Geometry check sheet. Reference: the model listing, model coordinates, mm. A direction names the side the tool comes from. Give positions to 0.01 mm unless a question says otherwise; leave off trailing zeros. Write each loop counter-clockwise with the first axis right and the second up, starting at its lowest first coordinate (ties: lowest second). Pieces come first, ordered by that corner, then holes. Notation, with made-up numbers: (9.25, -7.5) -> (49.25, -7.5) arc R27 ccw to (49.25, 9.5) -> close; hole circle Ø1 at (52.25, -9.75). An arc over 180 degrees is marked (long way). Write item = value, one per line. Start each with the question number.
1. Mould release check, pull along Y, two halves, no side actions. Record for faces 1 (the cylindrical face through (-2.994, 22.804, 4.93)), 2 (the flat face through (-14.07, -24.83, -7.4)), 3 (the flat face through (22.1, -7.3, 10)): pulls with the +Y half, pulls with the -Y half, needs draft (parallel to the pull), parting line crosses it, or undercut.
2. Depth check by flat-ended pin: P1, Ø12, axis at x = -9.5, z = -8, coming from the +Y side; P2, Ø14, axis at x = 11.5, y = -10.5, coming from the +Z side; P3, Ø3, axis at x = -12.5, z = 6.5, coming from the -Y side. Enter the tip coordinate at first touch or a pass-through.
3. Cross-section at C-C, the plane x = 16. Record the cut outline in (y, z), plus the area to 3 significant figures.
4. Cross-section at A-A, the plane z = 5.25. Record the cut outline in (x, y).
5. Cross-section at D-D, the plane z = -3.5. Record the cut outline in (x, y), plus the area to 3 significant figures.
6. Thickness scan on line 1 along Y through (x, z) = (0, 3.5); line 2 along X through (y, z) = (-13, 4.75); line 3 along Z through (x, y) = (0, 19). Record the ranges inside material, lowest first.
7. Set-up check for faces 4 (the flat face through (0, 0, 0)), 5 (the flat face through (-28.536, 0, -7)): record each of +Z, -Z, +X, -X, +Y, -Y from which the full face is reachable in a straight line by a thin tool's end or side.
8. Cross-section at B-B, the plane y = 10. Record the cut outline in (x, z), plus the area to 3 significant figures.
```python
from build123d import *

# Parameters (mm, degrees)
SKETCH1_R           = 25
SKETCH1_R_2         = 23
BOSS_EXTRUDE1_DEPTH = 10
BOSS_EXTRUDE2_DEPTH = 15


with BuildPart() as part:
    # Sketch1 → Boss-Extrude1 (new body)
    with BuildSketch(Plane.XY):
        Circle(SKETCH1_R)
        Circle(SKETCH1_R_2, mode=Mode.SUBTRACT)
    extrude(amount=BOSS_EXTRUDE1_DEPTH)

    # Sketch2 → Boss-Extrude2 (add)
    with BuildSketch(Plane(origin=(0, 0, 0), x_dir=(-1, 0, 0), z_dir=(0, 0, -1))):
        Polygon((0, 32.951018806), (-28.536419367, 16.475509403), (-28.536419367, -16.475509403), (0, -32.951018806), (28.536419367, -16.475509403), (28.536419367, 16.475509403), align=None)
    extrude(amount=BOSS_EXTRUDE2_DEPTH)


solid = part.part
```
Answers:
q1.face_1 = undercut
q1.face_2 = pulls with the -Y half
q1.face_3 = needs draft
q2.P1 = 30.93
q2.P2 = 0
q2.P3 = -22.45
q3.outline = (-23.71, -15) -> (23.71, -15) -> (23.71, 0) -> (19.21, 0) -> (19.21, 10) -> (16.52, 10) -> (16.52, 0) -> (-16.52, 0) -> (-16.52, 10) -> (-19.21, 10) -> (-19.21, 0) -> (-23.71, 0) -> close
q3.area = 765 mm^2
q4.outline = circle Ø50 at (0, 0); hole circle Ø46 at (0, 0)
q5.outline = (-28.54, -16.48) -> (0, -32.95) -> (28.54, -16.48) -> (28.54, 16.48) -> (0, 32.95) -> (-28.54, 16.48) -> close
q5.area = 2,820 mm^2
q6.line_1 = -25 to -23, 23 to 25
q6.line_2 = -21.35 to -18.97, 18.97 to 21.35
q6.line_3 = -15 to 0
q7.face_4 = +Z
q7.face_5 = +Z, -Z, -X, +Y, -Y
q8.outline = (-28.54, -15) -> (28.54, -15) -> (28.54, 0) -> (22.91, 0) -> (22.91, 10) -> (20.71, 10) -> (20.71, 0) -> (-20.71, 0) -> (-20.71, 10) -> (-22.91, 10) -> (-22.91, 0) -> (-28.54, 0) -> close
q8.area = 900 mm^2
